Read the model definition and answer for the solid it produces. Units are mm, in the model's axes. A direction names the side the tool comes from. Coordinates: 2 decimals unless noted, no trailing zeros. Write each loop counter-clockwise with the first axis right and the second up, starting at its lowest first coordinate (ties: lowest second). Pieces come first, ordered by that corner, then holes. Notation, with made-up numbers: (-5, 66.5) -> (3, 66.5) arc R21 ccw to (3, 97.5) -> close; hole circle Ø10 at (-30, 87.5). An arc over 180 degrees is marked (long way). Answer in a Markdown table with one row per item. Add a question column.
Item 1: Given pin 1 Ø2 at (y, z) = (-4.5, -7) entering from -X; pin 2 Ø3 at (y, z) = (-8, 1.5) entering from +X; pin 3 Ø1 at (x, y) = (-19.5, 17.5) entering from +Z; pin 4 Ø13 at (y, z) = (-18.5, -1) entering from -X, each flat-ended and moving along its own axis, determine where each tip first touches the part or whether it passes through.
Item 2: Section B-B on z = -6 is taken. Write down the section's boundary in (x, y) (3 decimals), then the cut area to 3 significant figures.
Item 3: For a pull along Z with two mould halves and no side action, classify faces 1 (the face through (-22, -2, 0)), 2 (the face through (22, -2, 0)), 3 (the face through (-11, -11, -15)), 4 (the face through (-0.5, -22, 0)) as +Z half, -Z half, draft (parallel to the pull), parting line (faces both ways), or undercut.
Item 4: Which of the six approach directions +Z, -Z, +X, -X, +Y, -Y give full straight-line access (tool end or side, diameter ignored) to faces 5 (the face through (7, 17, 15)), 6 (the face through (0.5, -22, 0))?
Item 5: Section A-A on z = 0 is taken. Write down the section's boundary in (x, y) (3 decimals), then the cut area to 3 significant figures.
Item 6: Section C-C on z = 8 is taken. Write down the section's boundary in (x, y) (3 decimals).
Item 7: Straight lines are drawn through the part: line 1 (Z direction, x = 22.75, y = 0); line 2 (X direction, y = 17.5, z = 5); line 3 (Y direction, x = -5, z = 2). For each, find the intervals that lie inside material, in ascending order. Write a range as from..to.
```python
from build123d import *

# Parameters (mm, degrees)
SKETCH2_W               = 1
SKETCH2_H               = 35
CUT_EXTRUDE1_DEPTH      = 39.405728739
CUT_EXTRUDE2_DEPTH      = 39.405728739
CUT_EXTRUDE2_DEPTH_BACK = 39.405728739
SKETCH3_R               = 2


with BuildPart() as part:
    # Sketch1 → Revolve1 (revolve)
    with BuildSketch(Plane(origin=(0, 0, 0), x_dir=(1, 0, 0), z_dir=(0, 1, 0))):
        with BuildLine():
            Line((17.9, -15), (16, -12))
            ThreePointArc((16, -12), (19.895478191, 2.042044945), (13.228756555, 15))
            Line((13.228756555, 15), (25, 15))
            Line((25, 15), (25, -15))
            Line((25, -15), (17.9, -15))
        make_face()
    revolve(axis=Axis((0, 0, -23.629385965), (0, 0, 1)))

    # Sketch2 → Cut-Extrude1 (cut, through all)
    with BuildSketch(Plane(origin=(0, 0, 0), x_dir=(1, 0, 0), z_dir=(0, 1, 0))):
        Rectangle(SKETCH2_W, SKETCH2_H)
    extrude(amount=-CUT_EXTRUDE1_DEPTH, mode=Mode.SUBTRACT)

    # Sketch3 → Cut-Extrude2 (cut, two sides: drawn at the far end of the back side and taken through both)
    with BuildSketch(Plane(origin=(0, 0, 0), x_dir=(0, 0, -1), z_dir=(1, 0, 0)).offset(-CUT_EXTRUDE2_DEPTH_BACK)):
        Circle(SKETCH3_R)
    extrude(amount=CUT_EXTRUDE2_DEPTH + CUT_EXTRUDE2_DEPTH_BACK, mode=Mode.SUBTRACT)


solid = part.part
```
Results below:
| question | item | result |
|---|---|---|
| 1 | pin 1 | stops at x = -24.75 |
| 1 | pin 2 | stops at x = 24.14 |
| 1 | pin 3 | passes through |
| 1 | pin 4 | stops at x = -21.93 |
| 2 | outline | (-0.5, -24.995) -> (-0.5, -19.072) arc R19.079 cw (long way) to (0.5, -19.072) -> (0.5, -24.995) arc R25 ccw (long way) to start |
| 2 | area | 814 mm2 |
| 3 | face 1 | undercut |
| 3 | face 2 | undercut |
| 3 | face 3 | -Z half |
| 3 | face 4 | draft |
| 4 | face 5 | +Z, +X, -X, +Y, -Y |
| 4 | face 6 | +Z, -Z, -Y |
| 5 | outline | (-24.92, -2) arc R25 ccw to (-0.5, -24.995) -> (-0.5, -19.994) arc R20 cw to (-19.9, -2) -> close; (-24.92, 2) -> (-19.9, 2) arc R20 cw to (19.9, 2) -> (24.92, 2) arc R25 ccw to start; (0.5, -24.995) arc R25 ccw to (24.92, -2) -> (19.9, -2) arc R20 cw to (0.5, -19.994) -> close |
| 5 | area | 662 mm2 |
| 6 | outline | (-0.5, -24.995) -> (-0.5, -18.323) arc R18.33 cw (long way) to (0.5, -18.323) -> (0.5, -24.995) arc R25 ccw (long way) to start |
| 7 | line 1 | z = -15..-2, 2..15 |
| 7 | line 2 | x = -17.85..-8.29, 8.29..17.85 |
| 7 | line 3 | y = -24.49..-19.26, 19.26..24.49 |
